Check sheet for the drawn part. Datum: minimum x, y, z corner. Units: mm. A direction names the side the tool comes from. Coordinates: 2 decimals unless noted, no trailing zeros. Loops run counter-clockwise (first coordinate to the right, second up) from the corner with the lowest first, then second, coordinate; pieces in that order, holes last. Notation, with made-up numbers: (-8.5, 26) - (18.5, 26) arc R21 cw to (18.5, 64) - close; hole circle Ø4 at (35, -16.5). An arc over 180 degrees is marked (long way). Write item = value, one per line. Start each with the question number.
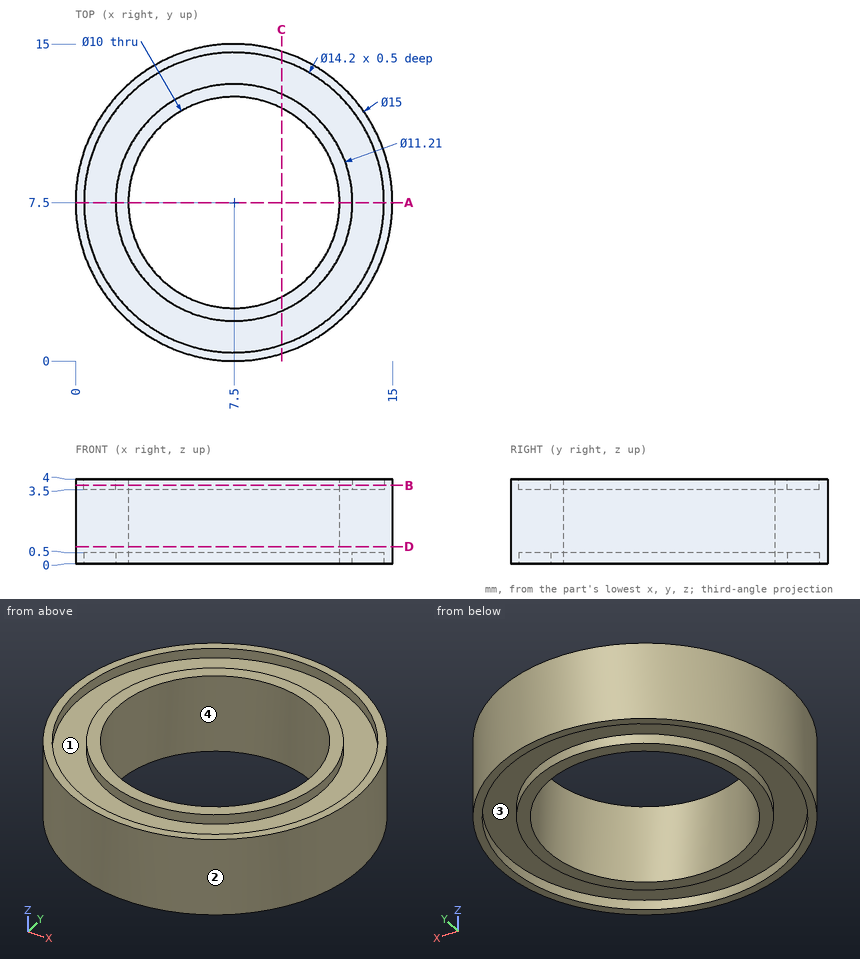
(1) Tool access check on the marked faces 3 and 4. Record the directions out of +Z, -Z, +X, -X, +Y, -Y that give a thin tool (end or side, any length) a straight path to the whole face; none if there is none.
(2) Draft check along Y on the marked faces 1 and 2. Enter one of: pulls with the +Y half, pulls with the -Y half, needs draft (parallel to the pull), parting line crosses it, or undercut.
(3) Sectioned sample at D-D on z = 0.8. Enter the section's corners in (x, y).
(4) Sectioned sample at B-B on z = 3.7. Enter the section's corners in (x, y) (3 decimals), plus the area to 3 significant figures.
(5) Depth check by flat-ended pin: pin 1 (3 mm diameter, centred on x = 12.5, y = 9, fed in from -Z). Enter the tip coordinate at first touch or a pass-through.
(6) Sectioned sample at C-C on x = 9.75. Enter the section's corners in (y, z).
(7) Sectioned sample at A-A on y = 7.5. Enter the section's corners in (x, z) (3 decimals).
(8) Scan lines: line 1 (Y direction, x = 7.5, z = 0.15) (3 decimals); line 2 (Y direction, x = 7.5, z = 1.6); line 3 (X direction, y = 10.75, z = 0.35). Record each from-to range of solid material in increasing order.
Working result:
q1.face_3 = -Z
q1.face_4 = +Z, -Z
q2.face_1 = undercut
q2.face_2 = parting line crosses it
q3.outline = circle Ø15 at (7.5, 7.5); hole circle Ø10 at (7.5, 7.5)
q4.outline = circle Ø15 at (7.5, 7.5); circle Ø11.21 at (7.5, 7.5); hole circle Ø14.2 at (7.5, 7.5); hole circle Ø10 at (7.5, 7.5)
q4.area = 38.5 mm2
q5.pin_1 = 0
q6.outline = (0.35, 0) - (0.77, 0) - (0.77, 0.5) - (2.37, 0.5) - (2.37, 0) - (3.03, 0) - (3.03, 4) - (2.37, 4) - (2.37, 3.5) - (0.77, 3.5) - (0.77, 4) - (0.35, 4) - close; (11.97, 0) - (12.63, 0) - (12.63, 0.5) - (14.23, 0.5) - (14.23, 0) - (14.65, 0) - (14.65, 4) - (14.23, 4) - (14.23, 3.5) - (12.63, 3.5) - (12.63, 4) - (11.97, 4) - close
q7.outline = (0, 0) - (0.4, 0) - (0.4, 0.5) - (1.895, 0.5) - (1.895, 0) - (2.5, 0) - (2.5, 4) - (1.895, 4) - (1.895, 3.5) - (0.4, 3.5) - (0.4, 4) - (0, 4) - close; (12.5, 0) - (13.105, 0) - (13.105, 0.5) - (14.6, 0.5) - (14.6, 0) - (15, 0) - (15, 4) - (14.6, 4) - (14.6, 3.5) - (13.105, 3.5) - (13.105, 4) - (12.5, 4) - close
q8.line_1 = 0 to 0.4, 1.895 to 2.5, 12.5 to 13.105, 14.6 to 15
q8.line_2 = 0 to 2.5, 12.5 to 15
q8.line_3 = 0.74 to 1.19, 2.93 to 3.7, 11.3 to 12.07, 13.81 to 14.26
